CAD build for the part. Positions are in the model's coordinates, mm. Round coordinates to 2 decimals unless told otherwise and drop trailing zeros. Order: outer loops, then holes, each group sorted by start corner. A loop starts at its lowest first (then second) coordinate and runs counter-clockwise, first axis right, second up. Notation, with made-up numbers: M 12,15 L 64,15 A20 ccw 64,30 Z; hole C -2,3 d7. An arc over 180 degrees is marked long. Answer as CSV lines item,"result". Start each with the question number.
```python
from build123d import *

# Parameters (mm, degrees)
SKETCH_1_W          = 100
SKETCH_1_H          = 90
EXTRUDE_1_DEPTH     = 4
SKETCH_2_R          = 4.5
CUT_EXTRUDE_1_DEPTH = 14


with BuildPart() as part:
    # 草图1 → 凸台-拉伸1 (new, symmetric)
    with BuildSketch(Plane.XY):
        Rectangle(SKETCH_1_W, SKETCH_1_H)
    extrude(amount=EXTRUDE_1_DEPTH, both=True)

    # 草图2 → 切除-拉伸1 (cut, symmetric)
    with BuildSketch(Plane.XY):
        with Locations((-35, -30)):
            Circle(SKETCH_2_R)
        with Locations((35, -30)):
            Circle(SKETCH_2_R)
        with Locations((-35, 30)):
            Circle(SKETCH_2_R)
        with Locations((35, 30)):
            Circle(SKETCH_2_R)
    extrude(amount=CUT_EXTRUDE_1_DEPTH, both=True, mode=Mode.SUBTRACT)


solid = part.part
```
Q1. Mould opens along X. For faces 1 (the flat face through (-50, -1, 0)), 2 (the flat face through (-1, 1, 4)), 3 (the cylindrical face through (-30.84, -31.72, 0.06)) say: +X half, -X half, draft (parallel to the pull), parting line (faces both ways), or undercut.
Q2. Band-saw the part on C-C, the plane x = -35. Write the cut outline in (y, z).
Q3. Band-saw the part on B-B, the plane z = -2. Write the cut outline in (x, y), then the cut area to 3 significant figures.
Q4. Probe line 1 along X through (y, z) = (-30, 0.25); line 2 along Y through (x, z) = (35, 1.5); line 3 along X through (y, z) = (26, 3.5). List the from-to ranges inside material, lowest first. Write a range as from..to.
Q5. Band-saw the part on A-A, the plane y = 30. Write the cut outline in (x, z).
Answer:
1,face 1,"-X half"
1,face 2,"draft"
1,face 3,"undercut"
2,outline,"M -45,-4 L -34.5,-4 L -34.5,4 L -45,4 Z; M -25.5,-4 L 25.5,-4 L 25.5,4 L -25.5,4 Z; M 34.5,-4 L 45,-4 L 45,4 L 34.5,4 Z"
3,outline,"M -50,-45 L 50,-45 L 50,45 L -50,45 Z; hole C -35,-30 d9; hole C -35,30 d9; hole C 35,-30 d9; hole C 35,30 d9"
3,area,"8,750 mm^2"
4,line 1,"x = -50..-39.5, -30.5..30.5, 39.5..50"
4,line 2,"y = -45..-34.5, -25.5..25.5, 34.5..45"
4,line 3,"x = -50..-37.06, -32.94..32.94, 37.06..50"
5,outline,"M -50,-4 L -39.5,-4 L -39.5,4 L -50,4 Z; M -30.5,-4 L 30.5,-4 L 30.5,4 L -30.5,4 Z; M 39.5,-4 L 50,-4 L 50,4 L 39.5,4 Z"
